Input: part model. Units: mm. Frame: model coordinates. Coordinates: 2 decimals unless noted, no trailing zeros. Write each loop counter-clockwise with the first axis right and the second up, starting at its lowest first coordinate (ties: lowest second). Pieces come first, ordered by that corner, then holes. Notation, with made-up numbers: M -34,48.25 L -13,48.25 A23 cw -13,68.25 Z; hole C 48,38 d6. An arc over 180 degrees is marked long. Answer as a JSON object with one key per item and string values. Group by question number.
from build123d import *

# Parameters (mm, degrees)
BOSS_EXTRUDE1_DEPTH = 8
CHAMFER1_SIZE       = 5


with BuildPart() as part:
    # Sketch1 → Boss-Extrude1 (new body)
    with BuildSketch(Plane.XY):
        Polygon((50, 65), (0, 65), (0, 0), (24.353078801, 0), (50, 55), align=None)
    extrude(amount=BOSS_EXTRUDE1_DEPTH)

    # Chamfer1
    chamfer1_edges = [part.edges().sort_by_distance(p)[0] for p in [
        (0, 65, 4),
    ]]
    chamfer(chamfer1_edges, length=CHAMFER1_SIZE)


solid = part.part
Q1. Pin query (flat end, axial travel): pin 1 Ø2 at (x, z) = (27, 2.5) entering from -Y; pin 2 Ø8 at (x, y) = (13, 13.5) entering from -Z. Return the tip coordinate at first contact, or that it passes through.
Q2. Section C-C, the plane x = 29.5. Return the cut outline in (y, z).
Q3. Section B-B, the plane y = 61. Return the cut outline in (x, z), and give its area (3 significant figures).
Q4. Line query: line 1 (X direction, y = 18, z = 2); line 2 (Y direction, x = 44.5, z = 0.75); line 3 (Y direction, x = 44, z = 2). Output: solid intervals per line, ascending. Write a range as from..to.
Q5. Section A-A, the plane z = 4. Return the cut outline in (x, y), and give its area (3 significant figures).
Filled in:
{
 "1": {"pin 1": "y = 3.53", "pin 2": "z = 0"},
 "2": {"outline": "M 11.04,0 L 65,0 L 65,8 L 11.04,8 Z"},
 "3": {"outline": "M 1,0 L 50,0 L 50,8 L 1,8 Z", "area": "392 mm^2"},
 "4": {"line 1": "0..32.75", "line 2": "43.21..65", "line 3": "42.13..65"},
 "5": {"outline": "M 0,0 L 24.35,0 L 50,55 L 50,65 L 5,65 L 0,60 Z", "area": "2,530 mm^2"}
}
